from build123d import *

# Parameters (mm, degrees)
SKETCH_1_W               = 20
SKETCH_1_H               = 20
SKETCH_1_R               = 1.94442565
EXTRUDE_1_DEPTH          = 25
CUT_EXTRUDE_1_DEPTH      = 52.961524227
PATTERN_CIRCULAR_1_COUNT = 4


with BuildPart() as part:
    # 草图1 → 凸台-拉伸1 (new, symmetric)
    with BuildSketch(Plane.XY):
        Rectangle(SKETCH_1_W, SKETCH_1_H)
        Circle(SKETCH_1_R, mode=Mode.SUBTRACT)
    extrude(amount=EXTRUDE_1_DEPTH, both=True)

    # 草图2 → 切除-拉伸1 (cut, symmetric)
    with BuildSketch(Plane.XY.offset(25)):
        Polygon((-32.933615203, 60.643738676), (-3.694439046, 10), (-2.5, 7.931170886), (2.5, 7.931170886), (3.694439046, 10), (32.933615203, 60.643738676), (32.933615203, 177.600443305), (-32.933615203, 177.600443305), align=None)
    cut_extrude_1 = extrude(amount=CUT_EXTRUDE_1_DEPTH, both=True, mode=Mode.SUBTRACT)

    # 阵列(圆周)1: 切除-拉伸1 ×4 about axis
    pattern_circular_1_axis = Axis((0, 0, 25), (0, 0, -1))
    for i in range(1, PATTERN_CIRCULAR_1_COUNT):
        add(cut_extrude_1.rotate(pattern_circular_1_axis, i * 360 / PATTERN_CIRCULAR_1_COUNT), mode=Mode.SUBTRACT)


solid = part.part
Can you work these out from the model? Positions are in its coordinate system, mm. A direction names the side the tool comes from. Round coordinates to 2 decimals unless told otherwise and drop trailing zeros. Write each loop counter-clockwise with the first axis right and the second up, starting at its lowest first coordinate (ties: lowest second). Pieces come first, ordered by that corner, then holes. Notation, with made-up numbers: (-16.5, -2.5) -> (34.5, -2.5) arc R21 ccw to (34.5, 31.5) -> close; hole circle Ø3 at (-5.5, 36). An arc over 180 degrees is marked (long way). One line per question, with ' | ' between items. Start each with the question number.
1) Suppose I cut it at D-D on x = -3. Write out the boundary of the cut face in (y, z).
2) If we mould it in two halves opening along Y, with no side actions, what happens to faces 5 (the flat face through (-8.98, -3.106, 0.35)), 6 (the flat face through (7, -10, 0)), 7 (the flat face through (3.09, 8.95, 0.35)), 8 (the flat face through (10, 7, 0))? For each: released by +Y, released by -Y, zero draft, split by the parting line, or undercut.
3) Suppose I cut it at A-A on x = 0. Write out the boundary of the cut face in (y, z), then the cut area to 3 significant figures.
4) Suppose I cut it at C-C on z = -1.5. Write out the boundary of the cut face in (x, y), then the cut area to 3 significant figures.
5) I need wall thicknesses on line 1 (Y direction, x = 0, z = -4.5); line 2 (X direction, y = 8.75, z = 16); line 3 (X direction, y = 1, z = 20.5). Which ranges of each line are inside material? Lowest first, please. Write a range as [from, to].
6) I'm going to push flat-ended pins straight in: P1, Ø5.5, axis at x = 0, z = 1, coming from the -Y side; P2, Ø1.5, axis at y = 1, z = -3.5, coming from the +X side; P3, Ø2.5, axis at y = -0.5, z = -10, coming from the -X side. Where does each tip first touch, or does it pass through?
7) On a 3-axis mill with a long thin cutter (end or side, diameter ignored), from which of +Z, -Z, +X, -X, +Y, -Y can I reach the whole of each face in a straight line? I mean faces 1 (the flat face through (8.98, 3.106, 0.35)), 2 (the flat face through (-8.95, 3.09, 0.35)), 3 (the flat face through (-3.106, 8.98, 0.35)), 4 (the flat face through (-3.09, -8.95, 0.35)). Say none if no direction works.
Return value:
1) outline: (-8.8, -25) -> (8.8, -25) -> (8.8, 25) -> (-8.8, 25) -> close
2) face 5: undercut | face 6: released by -Y | face 7: released by +Y | face 8: zero draft
3) outline: (-7.93, -25) -> (-1.94, -25) -> (-1.94, 25) -> (-7.93, 25) -> close; (1.94, -25) -> (7.93, -25) -> (7.93, 25) -> (1.94, 25) -> close | area: 599 mm2
4) outline: (-10, -10) -> (-3.69, -10) -> (-2.5, -7.93) -> (2.5, -7.93) -> (3.69, -10) -> (10, -10) -> (10, -3.69) -> (7.93, -2.5) -> (7.93, 2.5) -> (10, 3.69) -> (10, 10) -> (3.69, 10) -> (2.5, 7.93) -> (-2.5, 7.93) -> (-3.69, 10) -> (-10, 10) -> (-10, 3.69) -> (-7.93, 2.5) -> (-7.93, -2.5) -> (-10, -3.69) -> close; hole circle Ø3.89 at (0, 0) | area: 337 mm2
5) line 1: y = [-7.93, -1.94], [1.94, 7.93] | line 2: x = [-10, -2.97], [2.97, 10] | line 3: x = [-7.93, -1.67], [1.67, 7.93]
6) P1: stops at y = -8.36 | P2: stops at x = 7.93 | P3: stops at x = -7.93
7) face 1: +Z, -Z, +X | face 2: +Z, -Z, -X | face 3: +Z, -Z, +Y | face 4: +Z, -Z, -Y
